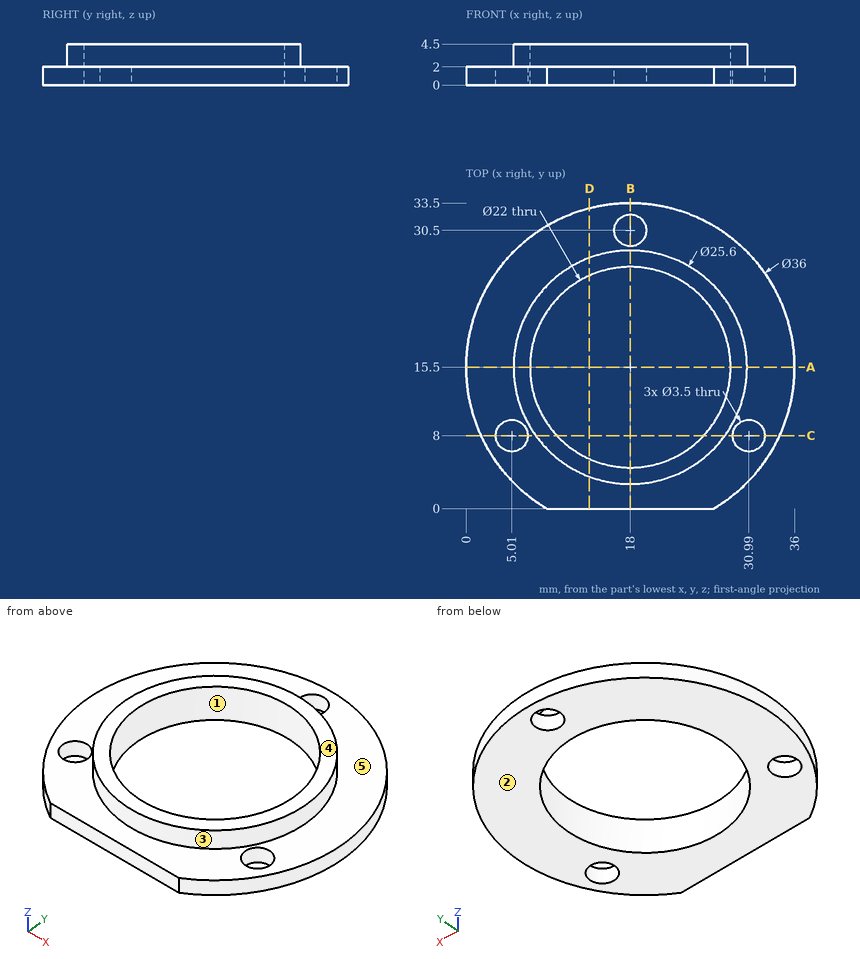
Could you check a few things on this drawing? It's one solid part, dimensions in mm from its lowest x, y, z. A direction names the side the tool comes from. Round coordinates to 2 decimals unless told otherwise and drop trailing zeros. Write each loop counter-clockwise with the first axis right and the second up, starting at its lowest first coordinate (ties: lowest second). Pieces come first, ordered by that corner, then holes. Notation, with made-up numbers: (43.25, 8.5) -> (87.25, 8.5) arc R12 cw to (87.25, 22.5) -> close; hole circle Ø9 at (61, 62.5). An arc over 180 degrees is marked (long way). Use a Markdown table: item, result.
1. Please list where these lines run through material, in increasing order: probe 1 along Y at (x, z) = (18, 3.55); probe 2 along Y at (x, z) = (28, 2.7) (1 decimal); probe 3 along X at (y, z) = (9.5, 0.4) (1 decimal).
Answer key:
| item | result |
|---|---|
| probe 1 | y = 2.7 to 4.5, 26.5 to 28.3 |
| probe 2 | y = 7.5 to 10.9, 20.1 to 23.5 |
| probe 3 | x = 1 to 4.1, 5.9 to 8.8, 27.2 to 30.1, 31.9 to 35 |
2. If we section it at B-B (x = 18): List the corners of the cut face in (y, z) for me, then the cut area to 3 significant figures.
Answer key:
| item | result |
|---|---|
| outline | (0, 0) -> (4.5, 0) -> (4.5, 4.5) -> (2.7, 4.5) -> (2.7, 2) -> (0, 2) -> close; (26.5, 0) -> (28.75, 0) -> (28.75, 2) -> (28.3, 2) -> (28.3, 4.5) -> (26.5, 4.5) -> close; (32.25, 0) -> (33.5, 0) -> (33.5, 2) -> (32.25, 2) -> close |
| area | 25.0 mm^2 |
3. For pin 1 Ø1.5 at (x, z) = (20.5, 1.5) entering from +Y (1 decimal); pin 2 Ø1.5 at (x, y) = (7, 25) entering from +Z; pin 3 Ø2 at (y, z) = (11.5, 4) entering from -X, each with a flat end and sliding along its axis, tell me the tip position at first contact or that it passes through.
Answer key:
| item | result |
|---|---|
| pin 1 | stops at y = 33.4 |
| pin 2 | stops at z = 2 |
| pin 3 | stops at x = 5.56 |
4. If we section it at D-D (x = 13.5): List the corners of the cut face in (y, z) for me.
Answer key:
| item | result |
|---|---|
| outline | (0, 0) -> (5.46, 0) -> (5.46, 4.5) -> (3.52, 4.5) -> (3.52, 2) -> (0, 2) -> close; (25.54, 0) -> (32.93, 0) -> (32.93, 2) -> (27.48, 2) -> (27.48, 4.5) -> (25.54, 4.5) -> close |
5. If we section it at C-C (y = 8): List the corners of the cut face in (x, z) for me.
Answer key:
| item | result |
|---|---|
| outline | (1.64, 0) -> (3.26, 0) -> (3.26, 2) -> (1.64, 2) -> close; (6.76, 0) -> (9.95, 0) -> (9.95, 4.5) -> (7.63, 4.5) -> (7.63, 2) -> (6.76, 2) -> close; (26.05, 0) -> (29.24, 0) -> (29.24, 2) -> (28.37, 2) -> (28.37, 4.5) -> (26.05, 4.5) -> close; (32.74, 0) -> (34.36, 0) -> (34.36, 2) -> (32.74, 2) -> close |
6. Which directions (+Z, -Z, +X, -X, +Y, -Y) give clear straight access to the entire face, cutting with the end or side of a thin tool? Please do the marked faces 4 and 5.
Answer key:
| item | result |
|---|---|
| face 4 | +Z, +X, -X, +Y, -Y |
| face 5 | +Z |
7. We'd pull the mould along X, two halves only. Please class the marked faces 1, 2 and 3: +X half, -X half, draft (parallel to the pull), parting line (faces both ways), or undercut.
Answer key:
| item | result |
|---|---|
| face 1 | undercut |
| face 2 | draft |
| face 3 | parting line |
8. If we section it at A-A (y = 15.5): List the corners of the cut face in (x, z) for me.
Answer key:
| item | result |
|---|---|
| outline | (0, 0) -> (7, 0) -> (7, 4.5) -> (5.2, 4.5) -> (5.2, 2) -> (0, 2) -> close; (29, 0) -> (36, 0) -> (36, 2) -> (30.8, 2) -> (30.8, 4.5) -> (29, 4.5) -> close |
